Verification items for the finished model (mm, model axes). A direction names the side the tool comes from. Round coordinates to 2 decimals unless told otherwise and drop trailing zeros. Write each loop counter-clockwise with the first axis right and the second up, starting at its lowest first coordinate (ties: lowest second). Pieces come first, ordered by that corner, then holes. Notation, with made-up numbers: (-20, 42) - (29, 42) arc R17 ccw to (29, 60) - close; hole circle Ø2 at (23, -24). An arc over 180 degrees is marked (long way). Answer as a JSON object with one key per item and string values. Group by question number.
1) Mould release check, pull along X, two halves, no side actions. Record for faces 1 (the cylindrical face through (4, 0, 3)), 2 (the flat face through (11, 3, 0)), 3 (the flat face through (14, 0, 0)): +X half, -X half, draft (parallel to the pull), parting line (faces both ways), or undercut.
2) Section check A-A (y = 0). Enter the section's corners in (x, z).
3) Section check C-C (y = -2.75). Enter the section's corners in (x, z).
4) Section check D-D (z = -2). Enter the section's corners in (x, y).
5) Set-up check for faces 4 (the cylindrical face through (5, 1, 0)), 5 (the cylindrical face through (9.99, -2.22, -1.15)), 6 (the flat face through (15, 0.5, 0)): record each of +Z, -Z, +X, -X, +Y, -Y from which the full face is reachable in a straight line by a thin tool's end or side.
6) Section check B-B (z = 0). Enter the section's corners in (x, y), then the cut area to 3 significant figures.
7) Go/stop test with flat-tipped pins: pin 1 Ø2 at (x, z) = (6.5, -3.5) entering from -Y; pin 2 Ø5 at (x, z) = (6, 2) entering from -Y; pin 3 Ø3 at (x, y) = (2.5, -2.5) entering from +Z; pin 4 Ø1 at (x, z) = (15, -0.5) entering from +Y. Record where each tip stops, or that it passes through.
8) Thickness scan on line 1 (Y direction, x = 3, z = 0); line 2 (Y direction, x = 10.1, z = 0); line 3 (Z direction, x = 12.5, y = -0.5). Record the ranges inside material, lowest first.
```python
from build123d import *

# Parameters (mm, degrees)
SKETCH1_R               = 3
BOSS_EXTRUDE1_DEPTH     = 9
SKETCH2_R               = 2.5
BOSS_EXTRUDE2_DEPTH     = 2
SKETCH3_R               = 4.5
BOSS_EXTRUDE3_DEPTH     = 5
CUT_EXTRUDE1_DEPTH      = 18.219175358
CUT_EXTRUDE1_DEPTH_BACK = 10.1
SKETCH4_R               = 1
CUT_EXTRUDE2_DEPTH      = 18.219175358
CUT_EXTRUDE2_DEPTH_BACK = 18.219175358
SKETCH6_R               = 1
CUT_EXTRUDE3_DEPTH      = 18.219175503
CUT_EXTRUDE3_DEPTH_BACK = 18.219175503
SKETCH7_W               = 4
SKETCH7_H               = 1


with BuildPart() as part:
    # Sketch1 → Boss-Extrude1 (new body)
    with BuildSketch(Plane(origin=(0, 0, 0), x_dir=(0, 0, -1), z_dir=(1, 0, 0))):
        Circle(SKETCH1_R)
    extrude(amount=BOSS_EXTRUDE1_DEPTH)

    # Sketch2 → Boss-Extrude2 (add)
    with BuildSketch(Plane(origin=(9, 0, 0), x_dir=(0, 0, -1), z_dir=(1, 0, 0))):
        Circle(SKETCH2_R)
    extrude(amount=BOSS_EXTRUDE2_DEPTH)

    # Sketch3 → Boss-Extrude3 (add)
    with BuildSketch(Plane(origin=(11, 0, 0), x_dir=(0, 0, -1), z_dir=(1, 0, 0))):
        Circle(SKETCH3_R)
    extrude(amount=BOSS_EXTRUDE3_DEPTH)

    # Sketch4 → Cut-Extrude1 (cut, two sides: drawn at the far end of the back side and taken through both)
    with BuildSketch(Plane.ZY.offset(-CUT_EXTRUDE1_DEPTH_BACK)):
        with Locations(Location((0, 0, 0), (0, 0, 180))):
            Circle(SKETCH4_R)
    extrude(amount=CUT_EXTRUDE1_DEPTH + CUT_EXTRUDE1_DEPTH_BACK, mode=Mode.SUBTRACT)

    # Sketch6 → Cut-Extrude2 (cut, two sides: drawn at the far end of the back side and taken through both)
    with BuildSketch(Plane.XY.offset(-CUT_EXTRUDE2_DEPTH_BACK)):
        with Locations(Location((10.1, 0, 0), (0, 0, 334.158067237))):
            Circle(SKETCH6_R)
    extrude(amount=CUT_EXTRUDE2_DEPTH + CUT_EXTRUDE2_DEPTH_BACK, mode=Mode.SUBTRACT)

    # Sketch7 → Cut-Extrude3 (cut, two sides: drawn at the far end of the back side and taken through both)
    with BuildSketch(Plane.XY.offset(-CUT_EXTRUDE3_DEPTH_BACK)):
        with Locations((16, 0)):
            Rectangle(SKETCH7_W, SKETCH7_H)
    extrude(amount=CUT_EXTRUDE3_DEPTH + CUT_EXTRUDE3_DEPTH_BACK, mode=Mode.SUBTRACT)


solid = part.part
```
Returned:
{
 "1": {"face 1": "draft", "face 2": "undercut", "face 3": "+X half"},
 "2": {"outline": "(0, -3) - (9, -3) - (9, -2.5) - (9.1, -2.5) - (9.1, -1) - (0, -1) - close; (0, 1) - (9.1, 1) - (9.1, 2.5) - (9, 2.5) - (9, 3) - (0, 3) - close; (11.1, -4.5) - (14, -4.5) - (14, 4.5) - (11.1, 4.5) - close"},
 "3": {"outline": "(0, -1.2) - (9, -1.2) - (9, 1.2) - (0, 1.2) - close; (11, -3.56) - (16, -3.56) - (16, 3.56) - (11, 3.56) - close"},
 "4": {"outline": "(0, -2.24) - (9, -2.24) - (9, -1.5) - (11, -1.5) - (11, -4.03) - (16, -4.03) - (16, -0.5) - (14, -0.5) - (14, 0.5) - (16, 0.5) - (16, 4.03) - (11, 4.03) - (11, 1.5) - (9, 1.5) - (9, 2.24) - (0, 2.24) - close; hole circle Ø2 at (10.1, 0)"},
 "5": {"face 4": "-X", "face 5": "none", "face 6": "+Z, -Z, +X"},
 "6": {"outline": "(0, -3) - (9, -3) - (9, -2.5) - (11, -2.5) - (11, -4.5) - (16, -4.5) - (16, -0.5) - (14, -0.5) - (14, 0.5) - (16, 0.5) - (16, 4.5) - (11, 4.5) - (11, 2.5) - (9, 2.5) - (9, 3) - (0, 3) - (0, 1) - (10.1, 1) arc R1 cw to (10.1, -1) - (0, -1) - close", "area": "85.2 mm2"},
 "7": {"pin 1": "y = -1.66", "pin 2": "y = -3", "pin 3": "z = 2.83", "pin 4": "y = 4.5"},
 "8": {"line 1": "-3 to -1, 1 to 3", "line 2": "-2.5 to -1, 1 to 2.5", "line 3": "-4.47 to 4.47"}
}
